```python
from build123d import *

# Parameters (mm, degrees)
SKETCH1_R           = 45
BOSS_EXTRUDE2_DEPTH = 200
SKETCH2_W           = 105
SKETCH2_H           = 318.049906591
CUT_EXTRUDE1_DEPTH  = 325.763563649
SKETCH3_R           = 50
BOSS_EXTRUDE3_DEPTH = 320
SKETCH4_R           = 25
CUT_EXTRUDE2_DEPTH  = 100
FILLET1_R           = 10


with BuildPart() as part:
    # Sketch1 → Boss-Extrude2 (new body)
    with BuildSketch(Plane.XY):
        with BuildLine():
            Line((140.402467833, -159.597532167), (-59.597532167, -159.597532167))
            Line((-59.597532167, -159.597532167), (-59.597532167, 40.402467833))
            ThreePointArc((-59.597532167, 40.402467833), (40.402467833, 140.402467833), (140.402467833, 40.402467833))
            Line((140.402467833, 40.402467833), (140.402467833, -159.597532167))
        make_face()
        with Locations((40.402467833, 40.402467833)):
            Circle(SKETCH1_R, mode=Mode.SUBTRACT)
    extrude(amount=BOSS_EXTRUDE2_DEPTH)

    # Sketch2 → Cut-Extrude1 (cut, through all)
    with BuildSketch(Plane(origin=(140.402467833, 0, 0), x_dir=(0, 0, -1), z_dir=(1, 0, 0))):
        with Locations((-100, 99.427421129)):
            Rectangle(SKETCH2_W, SKETCH2_H)
    extrude(amount=-CUT_EXTRUDE1_DEPTH, mode=Mode.SUBTRACT)

    # Sketch3 → Boss-Extrude3 (add)
    with BuildSketch(Plane.XZ.offset(159.597532167)):
        with Locations((40.402467833, 100)):
            Circle(SKETCH3_R)
    extrude(amount=BOSS_EXTRUDE3_DEPTH)

    # Sketch4 → Cut-Extrude2 (cut)
    with BuildSketch(Plane.XZ.offset(479.597532167)):
        with Locations((40.402467833, 100)):
            Circle(SKETCH4_R)
    extrude(amount=-CUT_EXTRUDE2_DEPTH, mode=Mode.SUBTRACT)

    # Fillet1
    fillet1_edges = [part.edges().sort_by_distance(p)[0] for p in [
        (-9.597532167, -159.597532167, 100),
    ]]
    fillet(fillet1_edges, radius=FILLET1_R)


solid = part.part
```
Geometry check sheet. Reference: the model listing, model coordinates, mm. A direction names the side the tool comes from. Give positions to 0.01 mm unless a question says otherwise; leave off trailing zeros. Order: outer loops, then holes, each group sorted by start corner. A loop starts at its lowest first (then second) coordinate and runs counter-clockwise, first axis right, second up.
1. Release check for a two-part mould opening along X. For faces 1 (the face through (34.54, 85.02, 175.92)), 2 (the face through (42, -7, 0)), 3 (the face through (-59.598, -83, 99)) record: pulls with the +X half, pulls with the -X half, needs draft (parallel to the pull), parting line crosses it, or undercut.
2. Thickness scan on L1, parallel to Z at x = 63, y = -39.5; L2, parallel to Y at x = 61, z = 115; L3, parallel to Y at x = 115.5, z = 86. Record the ranges inside material, lowest first.
3. Section check C-C, the plane z = 100. Enter the section's corners in (x, y), and give its area (3 significant figures).
4. Access from +Z, -Z, +X, -X, +Y, -Y to the whole of each face (thin tool, end or side, straight path). Record for faces 4 (the face through (38.2, 140.38, 23.42)), 5 (the face through (42, -59.598, 101)), 6 (the face through (86, -159.598, 143)).
5. Gauge pin test, flat ends, axial feed: pin 1 Ø6 at (x, z) = (53.5, 36) entering from +Y; pin 2 Ø15 at (x, z) = (47.5, 104) entering from -Y; pin 3 Ø10 at (x, z) = (45, 86) entering from +Y. Record the tip position at first contact, or that the pin passes through.
6. Section check D-D, the plane x = 108.5. Enter the section's corners in (y, z), and give its area (3 significant figures).
7. Section check A-A, the plane y = -28.5. Enter the section's corners in (x, z), and give its area (3 significant figures).
8. Section check B-B, the plane z = 169. Enter the section's corners in (x, y).
Values follow:
1. face 1: undercut
1. face 2: needs draft
1. face 3: pulls with the -X half
2. L1: z = 0 to 47.5, 152.5 to 200
2. L2: y = -479.6 to -59.6
2. L3: y = -159.6 to -59.6
3. outline: (-59.6, -159.6) - (-19.6, -159.6) arc R10 cw to (-9.6, -169.6) - (-9.6, -479.6) - (15.4, -479.6) - (15.4, -379.6) - (65.4, -379.6) - (65.4, -479.6) - (90.4, -479.6) - (90.4, -169.6) arc R10 cw to (100.4, -159.6) - (140.4, -159.6) - (140.4, -59.6) - (-59.6, -59.6) - close
3. area: 47,000 mm2
4. face 4: +Z, -Z, +Y
4. face 5: +X, -X, +Y
4. face 6: -Y
5. pin 1: stops at y = 139.89
5. pin 2: stops at y = -379.6
5. pin 3: stops at y = -59.6
6. outline: (-159.6, 0) - (113.63, 0) - (113.63, 47.5) - (-59.6, 47.5) - (-59.6, 152.5) - (113.63, 152.5) - (113.63, 200) - (-159.6, 200) - close
6. area: 36,500 mm2
7. outline: (-59.6, 0) - (140.4, 0) - (140.4, 47.5) - (-59.6, 47.5) - close; (-59.6, 152.5) - (140.4, 152.5) - (140.4, 200) - (-59.6, 200) - close
7. area: 19,000 mm2
8. outline: (-59.6, -159.6) - (140.4, -159.6) - (140.4, 40.4) arc R100 ccw to (-59.6, 40.4) - close; hole circle Ø90 at (40.4, 40.4)
